The figure shows three views and two pictorial views of one solid part (mm, origin at its lowest corner). Answer the questions. A direction names the side the tool comes from. Give positions to 0.01 mm unless a question says otherwise; leave off trailing zeros. Loops run counter-clockwise (first coordinate to the right, second up) from the corner with the lowest first, then second, coordinate; pieces in that order, holes last. Notation, with made-up numbers: M 40.5,59.5 L 90.5,59.5 A20 ccw 90.5,82.5 Z; hole C 66,-39 d6. An arc over 180 degrees is marked long. Answer as a JSON object with one key per item and string values. Group by question number.
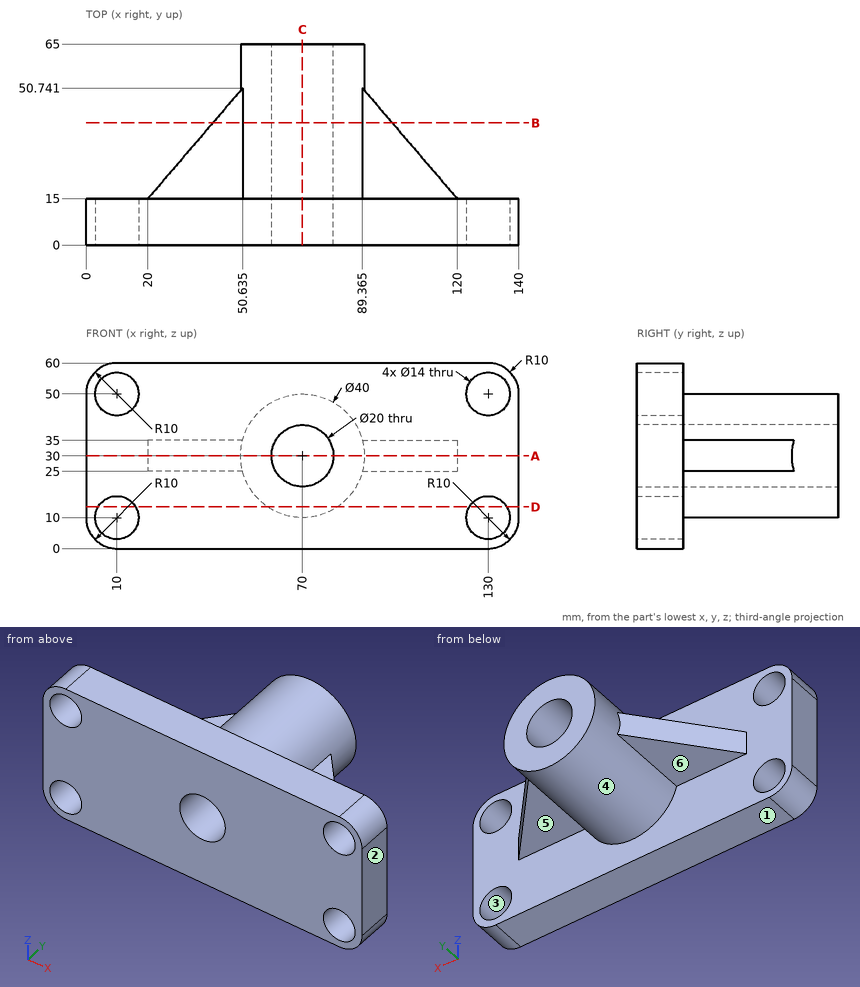
Item 1: A cutting plane is placed at D-D (z = 13.5). Determine the outline of the cut face in (x, y), and give its area (3 significant figures).
Item 2: A tool of negligible diameter and unlimited length cuts with its end or side. For the marked faces 4, 5 and 6, from which of +Z, -Z, +X, -X, +Y, -Y can it reach the whole face along a straight path? Write none if from no direction.
Item 3: Find the intervals of material crossed by probe 1 along X at (y, z) = (7, 50); probe 2 along Y at (x, z) = (70, 4.5); probe 3 along X at (y, z) = (8, 13), in increasing order. Write a range as [from, to].
Item 4: A cutting plane is placed at A-A (z = 30). Determine the outline of the cut face in (x, y).
Item 5: A cutting plane is placed at B-B (y = 39.5). Determine the outline of the cut face in (x, z) (3 decimals).
Item 6: A cutting plane is placed at C-C (x = 70). Determine the outline of the cut face in (y, z), and give its area (3 significant figures).
Item 7: Given pin 1 Ø15.5 at (x, y) = (30, 27) entering from +Z; pin 2 Ø8 at (y, z) = (45, 28) entering from +X; pin 3 Ø1 at (x, y) = (75.5, 21.5) entering from +Z (3 decimals), each flat-ended and moving along its own axis, determine where each tip first touches the part or whether it passes through.
Item 8: For a pull along X with two mould halves and no side action, classify the marked faces 1, 2 and 3 as pulls with the +X half, pulls with the -X half, needs draft (parallel to the pull), parting line crosses it, or undercut.
The answers:
{
 "1": {"outline": "M 0,0 L 3.94,0 L 3.94,15 L 0,15 Z; M 16.06,0 L 123.94,0 L 123.94,15 L 81.3,15 L 81.3,65 L 58.7,65 L 58.7,15 L 16.06,15 Z; M 136.06,0 L 140,0 L 140,15 L 136.06,15 Z", "area": "2,870 mm^2"},
 "2": {"face 4": "+Y", "face 5": "-Z, +X, +Y", "face 6": "-Z, -X, +Y"},
 "3": {"probe 1": "x = [0, 3], [17, 123], [137, 140]", "probe 2": "y = [0, 15]", "probe 3": "x = [0, 3.68], [16.32, 123.68], [136.32, 140]"},
 "4": {"outline": "M 0,0 L 60,0 L 60,65 L 50,65 L 50,50 L 20,15 L 0,15 Z; M 80,0 L 140,0 L 140,15 L 120,15 L 90,50 L 90,65 L 80,65 Z"},
 "5": {"outline": "M 41,25 L 50.635,25 A20 ccw 89.365,25 L 99,25 L 99,35 L 89.365,35 A20 ccw 50.635,35 L 41,35 Z; hole C 70,30 d20"},
 "6": {"outline": "M 0,0 L 15,0 L 15,10 L 65,10 L 65,20 L 0,20 Z; M 0,40 L 65,40 L 65,50 L 15,50 L 15,60 L 0,60 Z", "area": "1,600 mm^2"},
 "7": {"pin 1": "stops at z = 35", "pin 2": "stops at x = 97.71", "pin 3": "stops at z = 49.365"},
 "8": {"face 1": "needs draft", "face 2": "pulls with the +X half", "face 3": "undercut"}
}
